Verification items for the finished model (mm, model axes). Coordinates: 2 decimals unless noted, no trailing zeros. Write each loop counter-clockwise with the first axis right and the second up, starting at its lowest first coordinate (ties: lowest second). Pieces come first, ordered by that corner, then holes. Notation, with made-up numbers: (80.5, 27.25) -> (107.5, 27.25) arc R28 cw to (107.5, 57.25) -> close; hole circle Ø9 at (-37, -19.75). An arc over 180 degrees is marked (long way). Use CSV: the item, a comma, the result in double quotes.
```python
from build123d import *

# Parameters (mm, degrees)
SKETCH1_R           = 3
SKETCH1_R_2         = 2.5
BOSS_EXTRUDE1_DEPTH = 6
CHAMFER1_SIZE       = 0.2
SKETCH2_W           = 4.716397802
SKETCH2_H           = 0.1
CUT_EXTRUDE1_DEPTH  = 6


with BuildPart() as part:
    # Sketch1 → Boss-Extrude1 (new body)
    with BuildSketch(Plane.XY):
        Circle(SKETCH1_R)
        Circle(SKETCH1_R_2, mode=Mode.SUBTRACT)
    extrude(amount=BOSS_EXTRUDE1_DEPTH)

    # Chamfer1
    chamfer1_edges = [part.edges().sort_by_distance(p)[0] for p in [
        (-2.5, 0, 0),
        (-2.5, 0, 6),
    ]]
    chamfer(chamfer1_edges, length=CHAMFER1_SIZE)

    # Sketch2 → Cut-Extrude1 (cut)
    with BuildSketch(Plane.XY.offset(6)):
        with Locations((3, 0)):
            Rectangle(SKETCH2_W, SKETCH2_H)
    extrude(amount=-CUT_EXTRUDE1_DEPTH, mode=Mode.SUBTRACT)


solid = part.part
```
1) Cross-section at A-A (x = 0). Record the boundary of the cut face in (y, z).
Return value:
outline,"(-3, 0) -> (-2.7, 0) -> (-2.5, 0.2) -> (-2.5, 5.8) -> (-2.7, 6) -> (-3, 6) -> close; (2.5, 0.2) -> (2.7, 0) -> (3, 0) -> (3, 6) -> (2.7, 6) -> (2.5, 5.8) -> close"
2) Mould release check, pull along X, two halves, no side actions. Record for faces 1 (the cylindrical face through (-2.5, 0.1, 3)), 2 (the cylindrical face through (-3, 0, 3)): released by +X, released by -X, zero draft, split by the parting line, or undercut.
Return value:
face 1,"undercut"
face 2,"split by the parting line"
3) Gauge pin test, flat ends, axial feed: pin 1 (1 mm diameter, centred on x = 2.5, z = 2, fed in from -Y); pin 2 (3 mm diameter, centred on y = 1, z = 4, fed in from -X); pin 3 (0.6 mm diameter, centred on x = 2.5, z = 2.5, fed in from +Y). Record the tip position at first contact, or that the pin passes through.
Return value:
pin 1,"y = -2.24"
pin 2,"x = -3"
pin 3,"y = 2.04"
4) Cross-section at B-B (z = 0.85). Record the boundary of the cut face in (x, y).
Return value:
outline,"(2.5, -0.05) arc R2.5 cw (long way) to (2.5, 0.05) -> (3, 0.05) arc R3 ccw (long way) to (3, -0.05) -> close"
5) Scan lines: L1, parallel to Y at x = 0, z = 4.05; L2, parallel to X at y = 0, z = 2.2; L3, parallel to Y at x = 0.65, z = 5.6. Record each from-to range of solid material in increasing order.
Return value:
L1,"-3 to -2.5, 2.5 to 3"
L2,"-3 to -2.5"
L3,"-2.93 to -2.41, 2.41 to 2.93"
